For this review, take the finished solid that the model builds, in its own axes (mm). A direction names the side the tool comes from. Give positions to 0.01 mm unless a question says otherwise; leave off trailing zeros. Loops run counter-clockwise (first coordinate to the right, second up) from the corner with the lowest first, then second, coordinate; pieces in that order, holes last. Notation, with made-up numbers: (86.5, 44.5) -> (133.5, 44.5) arc R22 ccw to (133.5, 64.5) -> close; hole circle Ø11 at (31, -27). An arc over 180 degrees is marked (long way). One line per question, with ' | ' between items. Start each with the question number.
(1) Draft analysis for pull direction Z (two halves, no side actions). For faces 4 (the cylindrical face through (-2.17, -9.76, 222.66)), 5 (the flat face through (9, -4, 23)), 6 (the flat face through (0, -7, 428)), 7 (the flat face through (0, -8, 10)), state which applies: +Z half, -Z half, draft (parallel to the pull), parting line (faces both ways), or undercut.
(2) Wall thickness on probe 1 along Y at (x, z) = (0, 127.5); probe 2 along X at (y, z) = (0.5, 273); probe 3 along Y at (x, z) = (0, 22.55): over which ranges is each line inside the solid? List them lowest first.
(3) Consider section B-B (z = 89.5). Write out the cut boundary in (x, y), and give its area (3 significant figures).
(4) Insertion check: P1, Ø1.3, axis at y = 8.5, z = 7, coming from the +X side; P2, Ø1.5, axis at x = 0.5, z = 7, coming from the -Y side; P3, Ø0.5, axis at y = 9.5, z = 423, coming from the +X side. Each pin has a flat end and moves straight along its axis. Give the tip position at first contact, or say it passes through.
(5) Consider section A-A (y = 0). Write out the cut boundary in (x, z), and give its area (3 significant figures).
(6) Tool access review of faces 1 (the flat face through (9, -4, 22)), 2 (the cylindrical face through (-2.17, -9.76, 16.93)), 3 (the cylindrical face through (-2.059, -9.274, 4.93)): name each direction out of +Z, -Z, +X, -X, +Y, -Y from which nothing blocks a thin tool from reaching the whole face with its end or side.
from build123d import *

# Parameters (mm, degrees)
SKETCH1_R           = 9.5
SKETCH1_R_2         = 6
BOSS_EXTRUDE1_DEPTH = 10
CUT_EXTRUDE1_DEPTH  = 1.8
CUT_EXTRUDE2_START  = 1.8
CUT_EXTRUDE2_DEPTH  = 1.8
SKETCH4_R           = 9.75
SKETCH4_R_2         = 6
BOSS_EXTRUDE2_DEPTH = 2
SKETCH5_R           = 10
BOSS_EXTRUDE3_DEPTH = 10
SKETCH6_R           = 6
CUT_EXTRUDE3_DEPTH  = 27.153393745
SKETCH7_R           = 9.5
SKETCH7_R_2         = 6
BOSS_EXTRUDE4_DEPTH = 1
SKETCH8_R           = 10
SKETCH8_R_2         = 6
BOSS_EXTRUDE5_DEPTH = 6
SKETCH9_R           = 10
SKETCH9_R_2         = 6
BOSS_EXTRUDE6_DEPTH = 150
SKETCH10_R          = 10
SKETCH10_R_2        = 6
BOSS_EXTRUDE7_DEPTH = 223
SKETCH11_R          = 10
SKETCH11_R_2        = 6
BOSS_EXTRUDE8_DEPTH = 26
CUT_EXTRUDE4_DEPTH  = 1.8


with BuildPart() as part:
    # Sketch1 → Boss-Extrude1 (new body)
    with BuildSketch(Plane.XY):
        Circle(SKETCH1_R)
        Circle(SKETCH1_R_2, mode=Mode.SUBTRACT)
    extrude(amount=BOSS_EXTRUDE1_DEPTH)

    # Sketch2 → Cut-Extrude1 (cut)
    with BuildSketch(Plane(origin=(0, 9.5, 0), x_dir=(1, 0, 0), z_dir=(0, 1, 0))):
        with BuildLine():
            Line((1.5, -3.5), (1.5, -8.5))
            Line((1.5, -8.5), (1.5, -10))
            Line((1.5, -10), (-1.5, -10))
            Line((-1.5, -10), (-1.5, -8.5))
            Line((-1.5, -8.5), (-1.5, -3.5))
            ThreePointArc((-1.5, -3.5), (0, -2), (1.5, -3.5))
        make_face()
    extrude(amount=-CUT_EXTRUDE1_DEPTH, mode=Mode.SUBTRACT)

    # Sketch3 → Cut-Extrude2 (cut)
    with BuildSketch(Plane(origin=(0, -9.5, 0), x_dir=(1, 0, 0), z_dir=(0, 1, 0)).offset(CUT_EXTRUDE2_START)):
        with BuildLine():
            Line((1.5, -3.5), (1.5, -8.5))
            Line((1.5, -8.5), (1.5, -10.030894453))
            Line((1.5, -10.030894453), (-1.5, -10.030894453))
            Line((-1.5, -10.030894453), (-1.5, -8.5))
            Line((-1.5, -8.5), (-1.5, -3.5))
            ThreePointArc((-1.5, -3.5), (0, -2), (1.5, -3.5))
        make_face()
    extrude(amount=-CUT_EXTRUDE2_DEPTH, mode=Mode.SUBTRACT)

    # Sketch4 → Boss-Extrude2 (add)
    with BuildSketch(Plane.XY.offset(10)):
        Circle(SKETCH4_R)
        Circle(SKETCH4_R_2, mode=Mode.SUBTRACT)
    extrude(amount=BOSS_EXTRUDE2_DEPTH)

    # Sketch5 → Boss-Extrude3 (add)
    with BuildSketch(Plane.XY.offset(12)):
        Circle(SKETCH5_R)
    extrude(amount=BOSS_EXTRUDE3_DEPTH)

    # Sketch6 → Cut-Extrude3 (cut, through all)
    with BuildSketch(Plane.XY.offset(22)):
        Circle(SKETCH6_R)
    extrude(amount=-CUT_EXTRUDE3_DEPTH, mode=Mode.SUBTRACT)

    # Sketch7 → Boss-Extrude4 (add)
    with BuildSketch(Plane.XY.offset(22)):
        with Locations(Location((0, 0, 0), (0, 0, 260.915279713))):
            Circle(SKETCH7_R)
        Circle(SKETCH7_R_2, mode=Mode.SUBTRACT)
    extrude(amount=BOSS_EXTRUDE4_DEPTH)

    # Sketch8 → Boss-Extrude5 (add)
    with BuildSketch(Plane.XY.offset(23)):
        Circle(SKETCH8_R)
        Circle(SKETCH8_R_2, mode=Mode.SUBTRACT)
    extrude(amount=BOSS_EXTRUDE5_DEPTH)

    # Sketch9 → Boss-Extrude6 (add)
    with BuildSketch(Plane.XY.offset(29)):
        Circle(SKETCH9_R)
        Circle(SKETCH9_R_2, mode=Mode.SUBTRACT)
    extrude(amount=BOSS_EXTRUDE6_DEPTH)

    # Sketch10 → Boss-Extrude7 (add)
    with BuildSketch(Plane.XY.offset(179)):
        Circle(SKETCH10_R)
        Circle(SKETCH10_R_2, mode=Mode.SUBTRACT)
    extrude(amount=BOSS_EXTRUDE7_DEPTH)

    # Sketch11 → Boss-Extrude8 (add)
    with BuildSketch(Plane.XY.offset(402)):
        Circle(SKETCH11_R)
        Circle(SKETCH11_R_2, mode=Mode.SUBTRACT)
    extrude(amount=BOSS_EXTRUDE8_DEPTH)

    # Sketch12 → Cut-Extrude4 (cut)
    with BuildSketch(Plane(origin=(0, 10, 0), x_dir=(1, 0, 0), z_dir=(0, 1, 0))):
        with BuildLine():
            Line((1.5, -419.5), (1.5, -424.5))
            ThreePointArc((1.5, -424.5), (0, -426), (-1.5, -424.5))
            Line((-1.5, -424.5), (-1.5, -419.5))
            ThreePointArc((-1.5, -419.5), (0, -418), (1.5, -419.5))
        make_face()
    extrude(amount=-CUT_EXTRUDE4_DEPTH, mode=Mode.SUBTRACT)


solid = part.part
A:
1) face 4: draft | face 5: undercut | face 6: +Z half | face 7: undercut
2) probe 1: y = -10 to -6, 6 to 10 | probe 2: x = -9.99 to -5.98, 5.98 to 9.99 | probe 3: y = -9.5 to -6, 6 to 9.5
3) outline: circle Ø20 at (0, 0); hole circle Ø12 at (0, 0) | area: 201 mm^2
4) P1: stops at x = 5.35 | P2: stops at y = -7.7 | P3: stops at x = 3.8
5) outline: (-10, 12) -> (-9.75, 12) -> (-9.75, 10) -> (-9.5, 10) -> (-9.5, 0) -> (-6, 0) -> (-6, 428) -> (-10, 428) -> (-10, 23) -> (-9.5, 23) -> (-9.5, 22) -> (-10, 22) -> close; (6, 0) -> (9.5, 0) -> (9.5, 10) -> (9.75, 10) -> (9.75, 12) -> (10, 12) -> (10, 22) -> (9.5, 22) -> (9.5, 23) -> (10, 23) -> (10, 428) -> (6, 428) -> close | area: 3,410 mm^2
6) face 1: none | face 2: +Z, -Z | face 3: -Z
